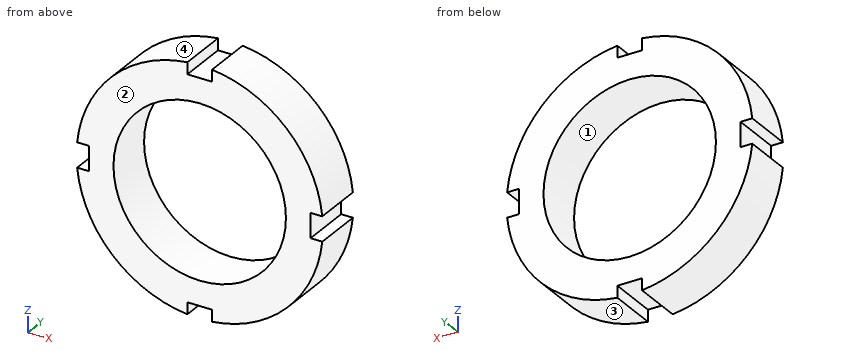
from build123d import *

# Parameters (mm, degrees)
SKETCH1_R           = 35
BOSS_EXTRUDE1_DEPTH = 20


with BuildPart() as part:
    # Sketch1 → Boss-Extrude1 (new body)
    with BuildSketch(Plane(origin=(0, 0, 0), x_dir=(1, 0, 0), z_dir=(0, 1, 0))):
        with BuildLine():
            Line((-5, 49.749371855), (-5, 45))
            Line((-5, 45), (5, 45))
            Line((5, 45), (5, 49.749371855))
            ThreePointArc((5, 49.749371855), (35.355339059, 35.355339059), (49.749371855, 5))
            Line((49.749371855, 5), (45, 5))
            Line((45, 5), (45, -5))
            Line((45, -5), (49.749371855, -5))
            ThreePointArc((49.749371855, -5), (35.355339059, -35.355339059), (5, -49.749371855))
            Line((5, -49.749371855), (5, -45))
            Line((5, -45), (-5, -45))
            Line((-5, -45), (-5, -49.749371855))
            ThreePointArc((-5, -49.749371855), (-35.355339059, -35.355339059), (-49.749371855, -5))
            Line((-49.749371855, -5), (-45, -5))
            Line((-45, -5), (-45, 5))
            Line((-45, 5), (-49.749371855, 5))
            ThreePointArc((-49.749371855, 5), (-35.355339059, 35.355339059), (-5, 49.749371855))
        make_face()
        with Locations(Location((0, 0, 0), (0, 0, 270))):
            Circle(SKETCH1_R, mode=Mode.SUBTRACT)
    extrude(amount=BOSS_EXTRUDE1_DEPTH)


solid = part.part
Input: part model. Units: mm. Frame: model coordinates. Face numbers are marked on the shaded views. Round coordinates to 2 decimals unless told otherwise and drop trailing zeros. Order: outer loops, then holes, each group sorted by start corner. A loop starts at its lowest first (then second) coordinate and runs counter-clockwise, first axis right, second up. Notation, with made-up numbers: (45, 60.5) - (66, 60.5) arc R28 cw to (66, 88.5) - close; hole circle Ø11 at (40.25, 38). An arc over 180 degrees is marked (long way). Use a Markdown table: item, result.
1. Section B-B on y = 6.75. Return the cut outline in (x, z).
Evaluation:
| item | result |
|---|---|
| outline | (-49.75, -5) arc R50 ccw to (-5, -49.75) - (-5, -45) - (5, -45) - (5, -49.75) arc R50 ccw to (49.75, -5) - (45, -5) - (45, 5) - (49.75, 5) arc R50 ccw to (5, 49.75) - (5, 45) - (-5, 45) - (-5, 49.75) arc R50 ccw to (-49.75, 5) - (-45, 5) - (-45, -5) - close; hole circle Ø70 at (0, 0) |
2. Section C-C on z = 0. Return the cut outline in (x, y).
Evaluation:
| item | result |
|---|---|
| outline | (-45, 0) - (-35, 0) - (-35, 20) - (-45, 20) - close; (35, 0) - (45, 0) - (45, 20) - (35, 20) - close |
3. Mould query, pull axis X, two halves, no side actions, for the marked faces 1, 2, 3 and 4. Classes: +X half, -X half, draft (parallel to the pull), parting line (faces both ways), or undercut.
Evaluation:
| item | result |
|---|---|
| face 1 | undercut |
| face 2 | draft |
| face 3 | +X half |
| face 4 | -X half |
4. Section D-D on x = 40. Return the cut outline in (y, z), then the cut area to 3 significant figures.
Evaluation:
| item | result |
|---|---|
| outline | (0, -30) - (20, -30) - (20, 30) - (0, 30) - close |
| area | 1,200 mm^2 |
5. First-contact query: pin 1 (12 mm diameter, centred on x = -9, y = 5.5, fed in from +Z); pin 2 (8 mm diameter, centred on x = 15, y = 13, fed in from +Z) (3 decimals); pin 3 (5 mm diameter, centred on y = 11.5, z = 47.5, fed in from -X). Flat tips, straight axial feed; report the tip coordinate or a pass-through.
Evaluation:
| item | result |
|---|---|
| pin 1 | z = 49.75 |
| pin 2 | z = 48.775 |
| pin 3 | x = -21.79 |
6. Material intervals for probe 1 along X at (y, z) = (9.5, 0); probe 2 along X at (y, z) = (15.5, 22.5); probe 3 along Z at (x, y) = (-30, 12.25), sorted ascending.
Evaluation:
| item | result |
|---|---|
| probe 1 | -45 to -35, 35 to 45 |
| probe 2 | -44.65 to -26.81, 26.81 to 44.65 |
| probe 3 | -40 to -18.03, 18.03 to 40 |
7. Section A-A on x = 0. Return the cut outline in (y, z).
Evaluation:
| item | result |
|---|---|
| outline | (0, -45) - (20, -45) - (20, -35) - (0, -35) - close; (0, 35) - (20, 35) - (20, 45) - (0, 45) - close |
